Read the model definition and answer for the solid it produces. Units are mm, in the model's axes. A direction names the side the tool comes from. Coordinates: 2 decimals unless noted, no trailing zeros. Loops run counter-clockwise (first coordinate to the right, second up) from the corner with the lowest first, then second, coordinate; pieces in that order, holes last. Notation, with made-up numbers: (-19.5, 69.25) -> (33.5, 69.25) arc R27 cw to (33.5, 95.25) -> close; hole circle Ø10 at (31, 30). An arc over 180 degrees is marked (long way). Answer as a JSON object with one key per item and string values. Group by question number.
Q1. The part is cut by section C-C on y = -2. Write down the section's boundary in (x, z).
Q2. Straight lines are drawn through the part: line 1 along X through (y, z) = (3, 14.5); line 2 along Z through (x, y) = (-50, -6); line 3 along X through (y, z) = (9, 9.25). For each, find the intervals that lie inside material, in ascending order. Write a range as [from, to].
Q3. The part is cut by section D-D on x = -35. Write down the section's boundary in (y, z), and give its area (3 significant figures).
Q4. Determine the mould class of faces 1 (the flat face through (-65, -1, 15)), 2 (the cylindrical face through (-30.754, -1.813, 14.79)), 3 (the flat face through (-50, -5, 20)) for opening direction Y: released by +Y, released by -Y, zero draft, split by the parting line, or undercut.
Q5. For faces 4 (the cylindrical face through (-54.292, -7.535, 13.648)), 5 (the cylindrical face through (-42.846, 2.605, 12.747)), determine the directions among +Z, -Z, +X, -X, +Y, -Y from which every point of the face is accessible in a straight line to the end or side of a thin tool.
Q6. The part is cut by section B-B on x = -50. Write down the section's boundary in (y, z).
Q7. The part is cut by section A-A on z = 15. Write down the section's boundary in (x, y).
from build123d import *

# Parameters (mm, degrees)
SKETCH_1_W                = 130
SKETCH_1_H                = 20
EXTRUDE_1_DEPTH           = 30
HOLE_WIZARD_1_D           = 9
HOLE_WIZARD_1_CBORE_D     = 15
HOLE_WIZARD_1_CBORE_DEPTH = 15
HOLE_WIZARD_M10_1_D       = 8.5
CHAMFER_1_SIZE            = 2
CHAMFER_2_SIZE            = 2


with BuildPart() as part:
    # 草图1 → 凸台-拉伸1 (new body)
    with BuildSketch(Plane.XY):
        Rectangle(SKETCH_1_W, SKETCH_1_H)
    extrude(amount=EXTRUDE_1_DEPTH)

    # 打孔尺寸(%根据)内六角圆柱头螺钉的类型1 (through all)
    with Locations(Plane(origin=(0, 10, 0), x_dir=(1, 0, 0), z_dir=(0, 1, 0))):
        with Locations((-50, -15), (50, -15)):
            CounterBoreHole(HOLE_WIZARD_1_D / 2, HOLE_WIZARD_1_CBORE_D / 2, HOLE_WIZARD_1_CBORE_DEPTH)

    # M10 螺纹孔1 (through all)
    with Locations(Plane.XY.offset(30)):
        with Locations((-35, -2), (35, -2)):
            Hole(HOLE_WIZARD_M10_1_D / 2)

    # 倒角1
    chamfer_1_edges = [part.edges().sort_by_distance(p)[0] for p in [
        (-65, 0, 30),
        (65, 0, 30),
        (-65, 0, 0),
        (65, 0, 0),
        (-65, 10, 15),
        (65, 10, 15),
    ]]
    chamfer(chamfer_1_edges, length=CHAMFER_1_SIZE)

    # 倒角2
    chamfer_2_edges = [part.edges().sort_by_distance(p)[0] for p in [
        (0, 10, 0),
    ]]
    chamfer(chamfer_2_edges, length=CHAMFER_2_SIZE)


solid = part.part
Final values:
{
 "1": {"outline": "(-65, 2) -> (-63, 0) -> (-39.25, 0) -> (-39.25, 30) -> (-63, 30) -> (-65, 28) -> close; (-30.75, 0) -> (30.75, 0) -> (30.75, 30) -> (-30.75, 30) -> close; (39.25, 0) -> (63, 0) -> (65, 2) -> (65, 28) -> (63, 30) -> (39.25, 30) -> close; hole circle Ø15 at (-50, 15); hole circle Ø15 at (50, 15)"},
 "2": {"line 1": "x = [-65, -57.48], [-42.52, 42.52], [57.48, 65]", "line 2": "z = [0, 10.5], [19.5, 30]", "line 3": "x = [-64, -54.82], [-45.18, 45.18], [54.82, 64]"},
 "3": {"outline": "(-10, 0) -> (-6.25, 0) -> (-6.25, 30) -> (-10, 30) -> close; (2.25, 0) -> (8, 0) -> (10, 2) -> (10, 30) -> (2.25, 30) -> close", "area": "343 mm2"},
 "4": {"face 1": "zero draft", "face 2": "undercut", "face 3": "released by +Y"},
 "5": {"face 4": "+Y, -Y", "face 5": "+Y"},
 "6": {"outline": "(-10, 0) -> (8, 0) -> (10, 2) -> (10, 7.5) -> (-5, 7.5) -> (-5, 10.5) -> (-10, 10.5) -> close; (-10, 19.5) -> (-5, 19.5) -> (-5, 22.5) -> (10, 22.5) -> (10, 30) -> (-10, 30) -> close"},
 "7": {"outline": "(-65, -10) -> (-54.5, -10) -> (-54.5, -5) -> (-57.5, -5) -> (-57.5, 10) -> (-63, 10) -> (-65, 8) -> close; (-45.5, -10) -> (45.5, -10) -> (45.5, -5) -> (42.5, -5) -> (42.5, 10) -> (-42.5, 10) -> (-42.5, -5) -> (-45.5, -5) -> close; (54.5, -10) -> (65, -10) -> (65, 8) -> (63, 10) -> (57.5, 10) -> (57.5, -5) -> (54.5, -5) -> close; hole circle Ø8.5 at (-35, -2); hole circle Ø8.5 at (35, -2)"}
}
